Read the model definition and answer for the solid it produces. Units are mm, in the model's axes. Face numbers are marked on the shaded views. A direction names the side the tool comes from. Coordinates: 2 decimals unless noted, no trailing zeros. Loops run counter-clockwise (first coordinate to the right, second up) from the corner with the lowest first, then second, coordinate; pieces in that order, holes last.
Q1. Section B-B (x = 0) is taken. Give the vertices of the cut face in (y, z).
Q2. Section A-A (z = 0) is taken. Give the vertices of the cut face in (x, y).
Q3. Straight lines are drawn through the part: line 1 (Y direction, x = -1, z = -5); line 2 (X direction, y = 9.75, z = 0); line 3 (Z direction, x = 2.5, y = 5.5). For each, find the intervals that lie inside material, in ascending order.
Q4. Flat-ended cylindrical pins translate along their axes: P1, Ø4, axis at y = 11.5, z = 1, coming from the -X side; P2, Ø1.5, axis at x = 3.5, y = 17, coming from the -Z side; P3, Ø3, axis at x = -5.5, y = 14.5, coming from the -Z side. Find the tip coordinate at first contact, or state that the pin passes through.
Q5. Section D-D (y = 21) is taken. Give the vertices of the cut face in (x, z), then the cut area to 3 significant figures.
Q6. Section C-C (y = 16.75) is taken. Give the vertices of the cut face in (x, z).
Q7. Which of the six approach directions +Z, -Z, +X, -X, +Y, -Y give full straight-line access (tool end or side, diameter ignored) to the marked faces 1 and 2?
from build123d import *

# Parameters (mm, degrees)
SKETCH2_R           = 5
BOSS_EXTRUDE1_DEPTH = 20
SKETCH3_R           = 7.5
BOSS_EXTRUDE2_DEPTH = 5
CHAMFER2_SIZE       = 0.5


with BuildPart() as part:
    # Sketch2 → Boss-Extrude1 (new body)
    with BuildSketch(Plane(origin=(0, 0, 0), x_dir=(1, 0, 0), z_dir=(0, 1, 0))):
        with Locations(Location((0, 0, 0), (0, 0, 270))):
            Circle(SKETCH2_R)
    extrude(amount=BOSS_EXTRUDE1_DEPTH)

    # Sketch3 → Boss-Extrude2 (add)
    with BuildSketch(Plane(origin=(0, 20, 0), x_dir=(1, 0, 0), z_dir=(0, 1, 0))):
        with Locations(Location((0, 0, 0), (0, 0, 270))):
            Circle(SKETCH3_R)
    extrude(amount=BOSS_EXTRUDE2_DEPTH)

    # Chamfer2
    chamfer2_edges = [part.edges().sort_by_distance(p)[0] for p in [
        (0, 0, -5),
        (0, 20, -7.5),
        (0, 25, -7.5),
    ]]
    chamfer(chamfer2_edges, length=CHAMFER2_SIZE)


solid = part.part
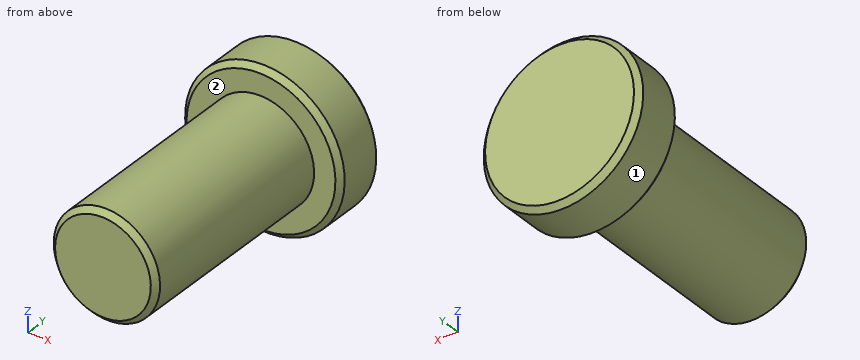
Numbers:
1. outline: (0, -4.5) - (0.5, -5) - (20, -5) - (20, -7) - (20.5, -7.5) - (24.5, -7.5) - (25, -7) - (25, 7) - (24.5, 7.5) - (20.5, 7.5) - (20, 7) - (20, 5) - (0.5, 5) - (0, 4.5) - close
2. outline: (-7.5, 20.5) - (-7, 20) - (-5, 20) - (-5, 0.5) - (-4.5, 0) - (4.5, 0) - (5, 0.5) - (5, 20) - (7, 20) - (7.5, 20.5) - (7.5, 24.5) - (7, 25) - (-7, 25) - (-7.5, 24.5) - close
3. line 1: y = 20 to 25
3. line 2: x = -5 to 5
3. line 3: z = -4.33 to 4.33
4. P1: stops at x = -5
4. P2: stops at z = -4.18
4. P3: stops at z = -3
5. outline: circle Ø15 at (0, 0)
5. area: 177 mm2
6. outline: circle Ø10 at (0, 0)
7. face 1: +Y, -Y
7. face 2: -Y
